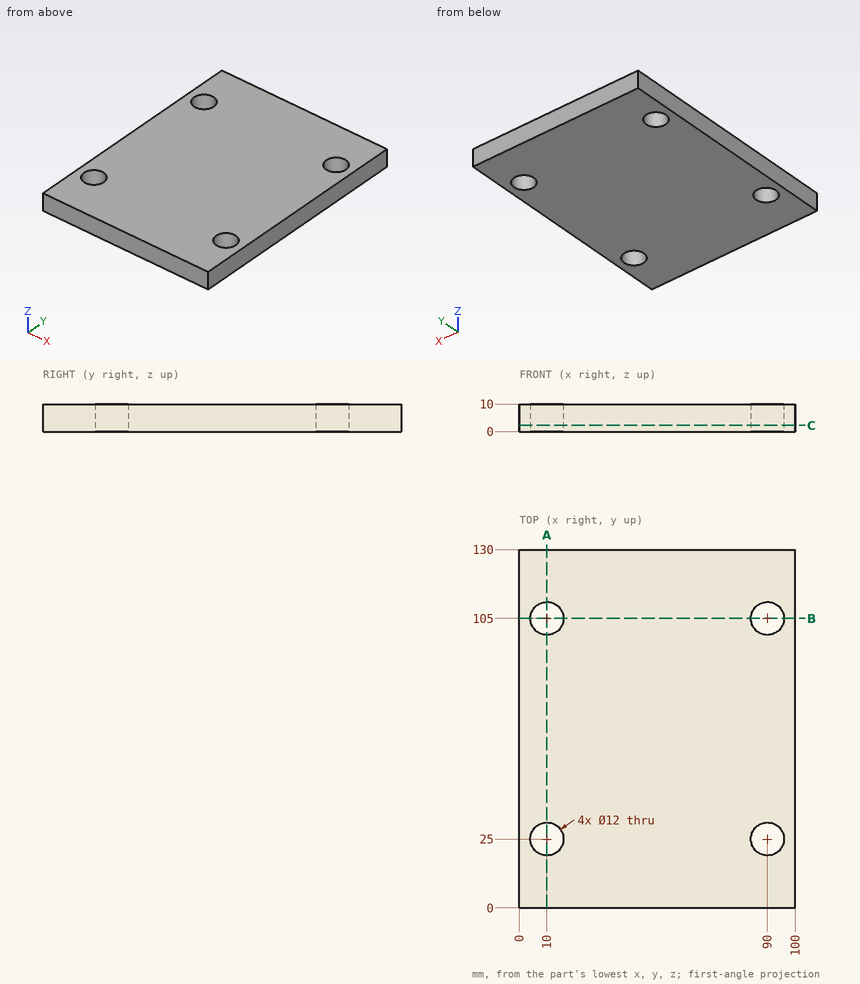
Check sheet for the drawn part. Datum: minimum x, y, z corner. Units: mm. Round coordinates to 2 decimals unless told otherwise and drop trailing zeros. Loops run counter-clockwise (first coordinate to the right, second up) from the corner with the lowest first, then second, coordinate; pieces in that order, holes last. Notation, with made-up numbers: (34, 10) - (38, 10) arc R24 cw to (38, 46) - close; hole circle Ø2 at (-26, -18.75). An arc over 180 degrees is marked (long way). Answer as a JSON object with one key per item and string values. Group by question number.
Q1. Sectioned sample at B-B, the plane y = 105. Enter the section's corners in (x, z).
Q2. Gauge pin test, flat ends, axial feed: P1, Ø6, axis at x = 46, y = 59, coming from the -Z side; P2, Ø9.5, axis at x = 90, y = 105, coming from the +Z side. Record the tip position at first contact, or that the pin passes through.
Q3. Sectioned sample at C-C, the plane z = 2.25. Enter the section's corners in (x, y), plus the area to 3 significant figures.
Q4. Scan lines: line 1 along Y through (x, z) = (10, 4.5); line 2 along Y through (x, z) = (85, 8.25); line 3 along X through (y, z) = (104, 5.75). Record each from-to range of solid material in increasing order. Write a range as [from, to].
Q5. Sectioned sample at A-A, the plane x = 10. Enter the section's corners in (y, z).
Solution:
{
 "1": {"outline": "(0, 0) - (4, 0) - (4, 10) - (0, 10) - close; (16, 0) - (84, 0) - (84, 10) - (16, 10) - close; (96, 0) - (100, 0) - (100, 10) - (96, 10) - close"},
 "2": {"P1": "stops at z = 0", "P2": "passes through"},
 "3": {"outline": "(0, 0) - (100, 0) - (100, 130) - (0, 130) - close; hole circle Ø12 at (10, 25); hole circle Ø12 at (10, 105); hole circle Ø12 at (90, 25); hole circle Ø12 at (90, 105)", "area": "12,500 mm²"},
 "4": {"line 1": "y = [0, 19], [31, 99], [111, 130]", "line 2": "y = [0, 21.68], [28.32, 101.68], [108.32, 130]", "line 3": "x = [0, 4.08], [15.92, 84.08], [95.92, 100]"},
 "5": {"outline": "(0, 0) - (19, 0) - (19, 10) - (0, 10) - close; (31, 0) - (99, 0) - (99, 10) - (31, 10) - close; (111, 0) - (130, 0) - (130, 10) - (111, 10) - close"}
}
